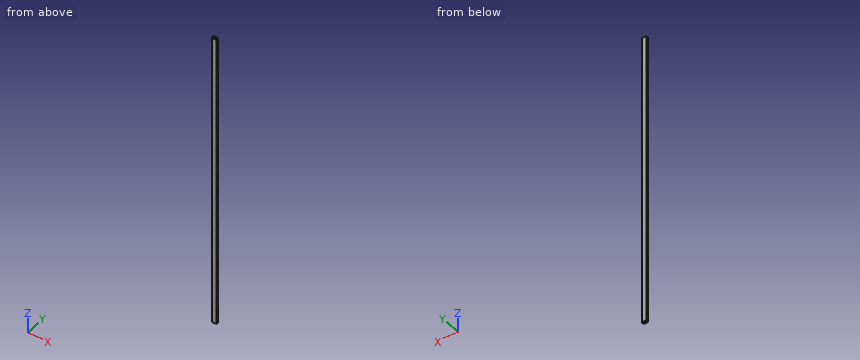
from build123d import *

# Parameters (mm, degrees)
SKETCH1_W           = 23
SKETCH1_H           = 13
SKETCH1_W_2         = 20
SKETCH1_H_2         = 10
EXTRUDE_THIN1_DEPTH = 1490


with BuildPart() as part:
    # Sketch1 → Extrude-Thin1 (new body)
    with BuildSketch(Plane.XY):
        with Locations((10, -5)):
            Rectangle(SKETCH1_W, SKETCH1_H)
        with Locations((10, -5)):
            Rectangle(SKETCH1_W_2, SKETCH1_H_2, mode=Mode.SUBTRACT)
    extrude(amount=EXTRUDE_THIN1_DEPTH)


solid = part.part
For this review, take the finished solid that the model builds, in its own axes (mm). Give positions to 0.01 mm unless a question says otherwise; leave off trailing zeros. Loops run counter-clockwise (first coordinate to the right, second up) from the corner with the lowest first, then second, coordinate; pieces in that order, holes last. Notation, with made-up numbers: (-20, 16.25) -> (-3, 16.25) arc R37 ccw to (-3, 54.25) -> close; hole circle Ø9 at (-26, 87.25). An arc over 180 degrees is marked (long way). One line per question, with ' | ' between items.
1) Insertion check: pin 1 Ø3 at (x, y) = (14.5, -2) entering from -Z. The pin has a flat end and moves straight along its axis. Give the tip position at first contact, or say it passes through.
Resolved:
pin 1: passes through
2) We need section B-B (z = 1094). Write out the cut boundary in (x, y), plus the area to 3 significant figures.
Resolved:
outline: (-1.5, -11.5) -> (21.5, -11.5) -> (21.5, 1.5) -> (-1.5, 1.5) -> close; hole (0, -10) -> (20, -10) -> (20, 0) -> (0, 0) -> close | area: 99.0 mm2
3) We need section A-A (y = -6.5). Write out the cut boundary in (x, z), plus the area to 3 significant figures.
Resolved:
outline: (-1.5, 0) -> (0, 0) -> (0, 1490) -> (-1.5, 1490) -> close; (20, 0) -> (21.5, 0) -> (21.5, 1490) -> (20, 1490) -> close | area: 4,470 mm2
4) To check wall thickness, follow probe 1 along Y at (x, z) = (16.75, 698.5); probe 2 along X at (y, z) = (-6.5, 498). State the ranges of each line that lie inside material, in increasing order.
Resolved:
probe 1: y = -11.5 to -10, 0 to 1.5 | probe 2: x = -1.5 to 0, 20 to 21.5
5) We need section C-C (x = 16). Write out the cut boundary in (y, z).
Resolved:
outline: (-11.5, 0) -> (-10, 0) -> (-10, 1490) -> (-11.5, 1490) -> close; (0, 0) -> (1.5, 0) -> (1.5, 1490) -> (0, 1490) -> close
